Here's how the part is built. I have some questions about the finished solid (model axes, mm). A direction names the side the tool comes from. Round coordinates to 2 decimals unless told otherwise and drop trailing zeros. Order: outer loops, then holes, each group sorted by start corner. A loop starts at its lowest first (then second) coordinate and runs counter-clockwise, first axis right, second up. Notation, with made-up numbers: M 54.25,3 L 83.25,3 A33 ccw 83.25,41 Z; hole C 2.25,45 d5. An arc over 180 degrees is marked long. Write item = value, one per line. Start each with the question number.
Item 1: I want a section at A-A, the plane y = -37. List the corners of the cut face in (x, z) for me, plus the area to 3 significant figures.
Item 2: We'd pull the mould along X, two halves only. Please class faces 1 (the face through (-85, 135.747, -3)), 2 (the face through (-68.634, -1.4, -5.42)), 3 (the face through (-93, -61.253, 0)): pulls with the +X half, pulls with the -X half, needs draft (parallel to the pull), parting line crosses it, or undercut.
Item 3: For faces 4 (the face through (-93, -64.253, 0)), 5 (the face through (-114.852, -2.205, -2.864)), which set-ups out of +Z, -Z, +X, -X, +Y, -Y let a thin tool reach every point of the face, with its end or its side?
Item 4: Please list where these lines run through material, in increasing order: L1, parallel to X at y = 5, z = 0; L2, parallel to X at y = -35.5, z = -5 (3 decimals); L3, parallel to Y at x = -88.5, z = -2.
Item 5: I'm going to push flat-ended pins straight in: P1, Ø12, axis at x = -87, y = 79, coming from the +Z side; P2, Ø10, axis at y = 72.5, z = 11, coming from the +X side; P3, Ø3, axis at y = 37.5, z = -17.5, coming from the +X side. Where does each tip first touch, or does it pass through?
```python
from build123d import *

# Parameters (mm, degrees)
SHELL1_T  = -3
FILLET1_R = 5
FILLET2_R = 1


with BuildPart() as part:
    # Sketch1 → Revolve1 (revolve)
    with BuildSketch(Plane.XY, mode=Mode.PRIVATE) as revolve1_sk:
        with BuildLine():
            Line((-93.039279644, 135.747175363), (-93.039279644, -64.252824637))
            Line((-93.039279644, -64.252824637), (-118.039279644, -64.252824637))
            Line((-118.039279644, -64.252824637), (-118.039279644, 55.747175363))
            add(Edge.make_bspline(
                [(-118.039279644, 55.747175363), (-103.478005536, 95.090899145), (-103.039279644, 135.747175363)],
                knots=[0, 0, 0, 0.941503214, 0.941503214, 0.941503214], degree=2))
            Line((-103.039279644, 135.747175363), (-93.039279644, 135.747175363))
        make_face()
    revolve(revolve1_sk.sketch.rotate(Axis((-93.039279644, 135.747175363, 0), (0, -1, 0)), 270), axis=Axis((-93.039279644, 135.747175363, 0), (0, -1, 0)))

    # Shell1
    shell1_openings = [part.faces().sort_by_distance(p)[0] for p in [
        (-93.039279644, 135.747175363, 0),
    ]]
    offset(amount=SHELL1_T, openings=shell1_openings, kind=Kind.INTERSECTION)

    # Fillet1
    fillet1_edges = [part.edges().sort_by_distance(p)[0] for p in [
        (-93.039279644, 55.747175363, -25),
        (-93.039279644, -64.252824637, -25),
    ]]
    fillet(fillet1_edges, radius=FILLET1_R)

    # Fillet2
    fillet2_edges = [part.edges().sort_by_distance(p)[0] for p in [
        (-93.039279644, 135.747175363, -6.999825357),
        (-93.039279644, 135.747175363, -10),
    ]]
    fillet(fillet2_edges, radius=FILLET2_R)


solid = part.part
```
Filled in:
q1.outline = C -93.04,0 d50; hole C -93.04,0 d44
q1.area = 443 mm^2
q2.face_1 = needs draft
q2.face_2 = parting line crosses it
q2.face_3 = undercut
q3.face_4 = +Z, -Z, +X, -X, -Y
q3.face_5 = none
q4.L1 = -118.04 to -115.04, -71.04 to -68.04
q4.L2 = -117.534 to -114.464, -71.615 to -68.544
q4.L3 = -64.25 to -61.25
q5.P1 = 18.84
q5.P2 = -73.92
q5.P3 = -73.83
